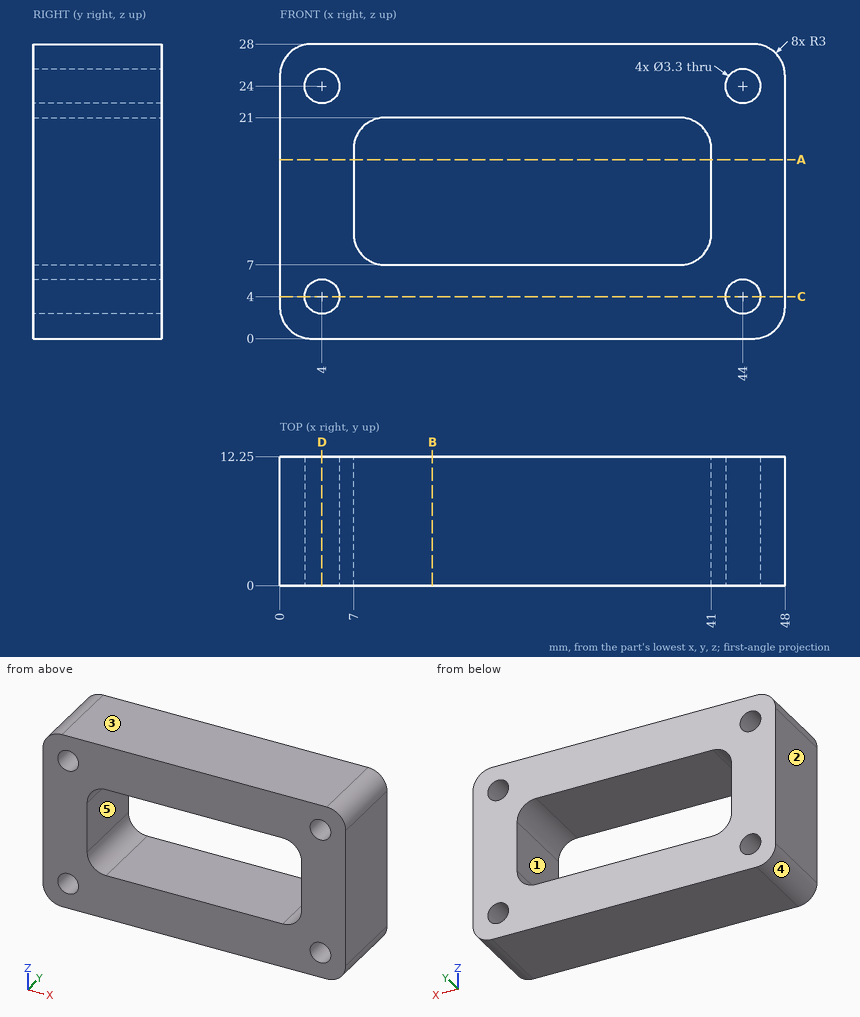
Print and shaded views of the part. All mm, measured from the part's lowest x, y and z. A direction names the side the tool comes from. Coordinates: 2 decimals unless noted, no trailing zeros. Loops run counter-clockwise (first coordinate to the right, second up) from the corner with the lowest first, then second, coordinate; pieces in that order, holes last. Notation, with made-up numbers: M -10.5,29.25 L 29.5,29.25 A27 ccw 29.5,59.25 Z; hole C -24,86 d1. An arc over 180 degrees is marked long. Use a Markdown table: item, result. Add a question column.
Q1. Cut at C-C (z = 4). Write the cut outline in (x, y), and give its area (3 significant figures).
Q2. Cut at A-A (z = 17). Write the cut outline in (x, y), and give its area (4 significant figures).
Q3. Which spindle directions (+Z, -Z, +X, -X, +Y, -Y) get a long thin tool onto all of the face, cutting with end or side? Do the marked faces 4 and 5. Say none if no direction does.
Q4. Mould opens along X. For the marked faces 1, 2 and 3 say: +X half, -X half, draft (parallel to the pull), parting line (faces both ways), or undercut.
Q5. Probe L1, parallel to X at y = 5, z = 4; L2, parallel to X at y = 8.5, z = 11.75; L3, parallel to X at y = 7, z = 22.5. List the from-to ranges inside material, lowest first.
Q6. Cut at B-B (x = 14.5). Write the cut outline in (y, z), and give its area (4 significant figures).
Q7. Cut at D-D (x = 4). Write the cut outline in (y, z).
Worked out:
| question | item | result |
|---|---|---|
| 1 | outline | M 0,0 L 2.35,0 L 2.35,12.25 L 0,12.25 Z; M 5.65,0 L 42.35,0 L 42.35,12.25 L 5.65,12.25 Z; M 45.65,0 L 48,0 L 48,12.25 L 45.65,12.25 Z |
| 1 | area | 507 mm2 |
| 2 | outline | M 0,0 L 7,0 L 7,12.25 L 0,12.25 Z; M 41,0 L 48,0 L 48,12.25 L 41,12.25 Z |
| 2 | area | 171.5 mm2 |
| 3 | face 4 | -Z, -X, +Y, -Y |
| 3 | face 5 | +Y, -Y |
| 4 | face 1 | undercut |
| 4 | face 2 | -X half |
| 4 | face 3 | draft |
| 5 | L1 | x = 0 to 2.35, 5.65 to 42.35, 45.65 to 48 |
| 5 | L2 | x = 0 to 7, 41 to 48 |
| 5 | L3 | x = 0 to 3.31, 4.69 to 43.31, 44.69 to 48 |
| 6 | outline | M 0,0 L 12.25,0 L 12.25,7 L 0,7 Z; M 0,21 L 12.25,21 L 12.25,28 L 0,28 Z |
| 6 | area | 171.5 mm2 |
| 7 | outline | M 0,0 L 12.25,0 L 12.25,2.35 L 0,2.35 Z; M 0,5.65 L 12.25,5.65 L 12.25,22.35 L 0,22.35 Z; M 0,25.65 L 12.25,25.65 L 12.25,28 L 0,28 Z |
